Check sheet for the drawn part. Datum: minimum x, y, z corner. Units: mm. Round coordinates to 2 decimals unless told otherwise and drop trailing zeros. Order: outer loops, then holes, each group sorted by start corner. A loop starts at its lowest first (then second) coordinate and runs counter-clockwise, first axis right, second up.
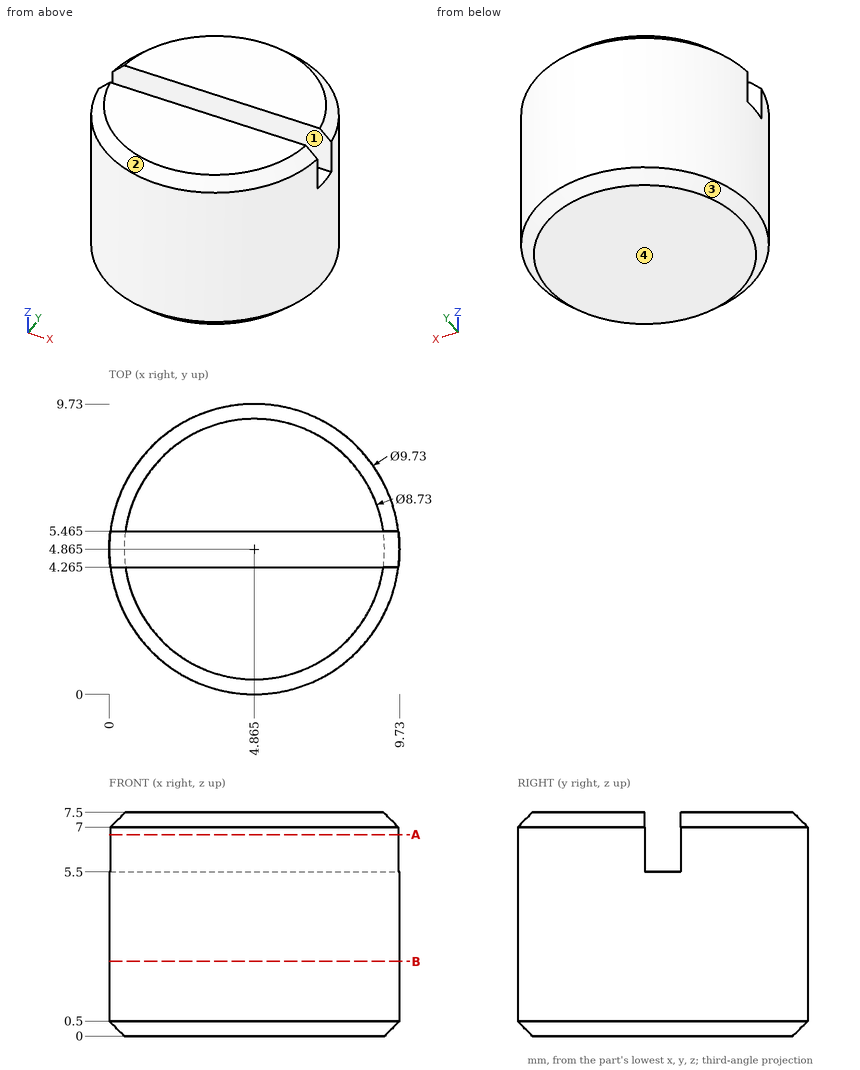
(1) Sectioned sample at B-B, the plane z = 2.5. Record the cut outline in (x, y) (3 decimals).
Returned:
outline: circle Ø9.73 at (4.865, 4.865)
(2) Sectioned sample at A-A, the plane z = 6.75. Record the cut outline in (x, y) (3 decimals), and give its area (3 significant figures).
Returned:
outline: (0.037, 4.265) arc R4.865 ccw to (9.693, 4.265) - close; (0.037, 5.465) - (9.693, 5.465) arc R4.865 ccw to start
area: 62.7 mm2
(3) Material ranges on line 1 (Y direction, x = 4.25, z = 6.5) (3 decimals); line 2 (Z direction, x = 7, y = 5); line 3 (Y direction, x = 4, z = 1.25), recorded low to high.
Returned:
line 1: y = 0.039 to 4.265, 5.465 to 9.691
line 2: z = 0 to 5.5
line 3: y = 0.08 to 9.65
(4) Draft check along Y on the marked faces 1, 2, 3 and 4. Enter one of: released by +Y, released by -Y, zero draft, split by the parting line, or undercut.
Returned:
face 1: undercut
face 2: released by -Y
face 3: split by the parting line
face 4: zero draft
(5) Depth check by flat-ended pin: P1, Ø3, axis at y = 2, z = 4, coming from the +X side; P2, Ø1, axis at x = 5.5, z = 7, coming from the +Y side. Enter the tip coordinate at first touch or a pass-through.
Returned:
P1: stops at x = 9.53
P2: stops at y = 9.73
